Build history of the part. All positions in model axes, mm. Round coordinates to 2 decimals unless told otherwise and drop trailing zeros. Write each loop counter-clockwise with the first axis right and the second up, starting at its lowest first coordinate (ties: lowest second). Pieces come first, ordered by that corner, then holes.
1) Flat gauge pins, fed straight in: pin 1 (5 mm diameter, centred on y = -2, z = -43.5, fed in from -X); pin 2 (0.7 mm diameter, centred on x = 13, z = 60, fed in from -Y); pin 3 (0.5 mm diameter, centred on y = 13, z = -76.5, fed in from -X); pin 4 (2 mm diameter, centred on y = 0.5, z = -88, fed in from -X). Where does each tip first touch, or does it go through?
2) Saw through at A-A (x = 0). Write the cut outline in (y, z), plus the area to 3 significant figures.
3) Wall check: probe 1 along X at (y, z) = (0, -110.5); probe 2 along X at (y, z) = (-8, -33); probe 3 along Y at (x, z) = (8.25, 47.5). Give the ranges that are in metal, low to high.
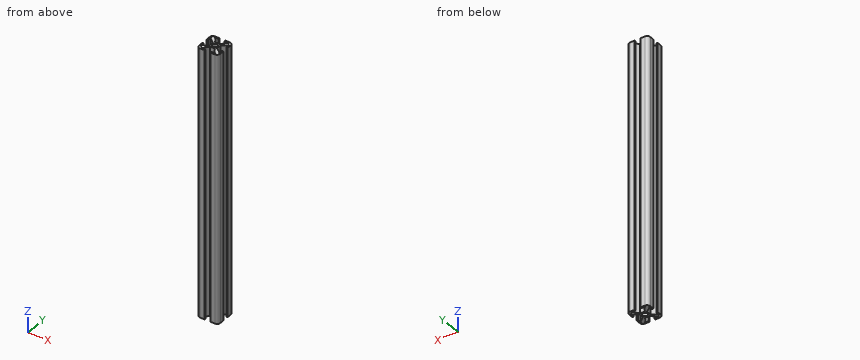
from build123d import *

# Parameters (mm, degrees)
SKETCH_1_W               = 30
SKETCH_1_H               = 30
EXTRUDE_1_DEPTH          = 190
FILLET_1_R               = 4.5
SKETCH_2_W               = 8.2
SKETCH_2_H               = 0.3
SKETCH_2_H_2             = 1.9
SKETCH_2_R               = 3.4
CUT_EXTRUDE_1_DEPTH      = 381.59164468
PATTERN_CIRCULAR_1_COUNT = 4


with BuildPart() as part:
    # 草图1 → 凸台-拉伸1 (new, symmetric)
    with BuildSketch(Plane.XY):
        Rectangle(SKETCH_1_W, SKETCH_1_H)
    extrude(amount=EXTRUDE_1_DEPTH, both=True)

    # 圆角1
    fillet_1_edges = [part.edges().sort_by_distance(p)[0] for p in [
        (-15, 15, 0),
        (15, 15, 0),
        (15, -15, 0),
        (-15, -15, 0),
    ]]
    fillet(fillet_1_edges, radius=FILLET_1_R)

    # 草图2 → 切除-拉伸1 (cut, through all)
    with BuildSketch(Plane.XY.offset(190)):
        with Locations((0, 12.95)):
            Rectangle(SKETCH_2_W, SKETCH_2_H)
        with Locations((0, 14.05)):
            Rectangle(SKETCH_2_W, SKETCH_2_H_2)
        Polygon((10.25, 13.1), (4.1, 13.1), (4.1, 12.8), (-4.1, 12.8), (-4.1, 13.1), (-10.25, 13.1), (-10.25, 12.5), (-8.429704265, 12.5), (8.429704265, 12.5), (10.25, 12.5), align=None)
        Polygon((3.479704265, 5.3), (8.429704265, 12.5), (-8.429704265, 12.5), (-3.479704265, 5.3), align=None)
        Circle(SKETCH_2_R)
    cut_extrude_1 = extrude(amount=-CUT_EXTRUDE_1_DEPTH, mode=Mode.SUBTRACT)

    # 阵列(圆周)1: 切除-拉伸1 ×4 about axis
    pattern_circular_1_axis = Axis((0, 0, 0), (0, 0, 1))
    for i in range(1, PATTERN_CIRCULAR_1_COUNT):
        add(cut_extrude_1.rotate(pattern_circular_1_axis, i * 360 / PATTERN_CIRCULAR_1_COUNT), mode=Mode.SUBTRACT)


solid = part.part
Evaluation:
1. pin 1: stops at x = -15
1. pin 2: stops at y = -14.45
1. pin 3: stops at x = -14.4
1. pin 4: stops at x = -5.3
2. outline: (-5.3, -190) - (-3.4, -190) - (-3.4, 190) - (-5.3, 190) - close; (3.4, -190) - (5.3, -190) - (5.3, 190) - (3.4, 190) - close
2. area: 1,440 mm2
3. probe 1: x = -5.3 to -3.4, 3.4 to 5.3
3. probe 2: x = -15 to -13.1, -11.87 to -5.34, 5.34 to 11.87, 13.1 to 15
3. probe 3: y = -15 to -13.1, -12.24 to -5.51, 5.51 to 12.24, 13.1 to 15
